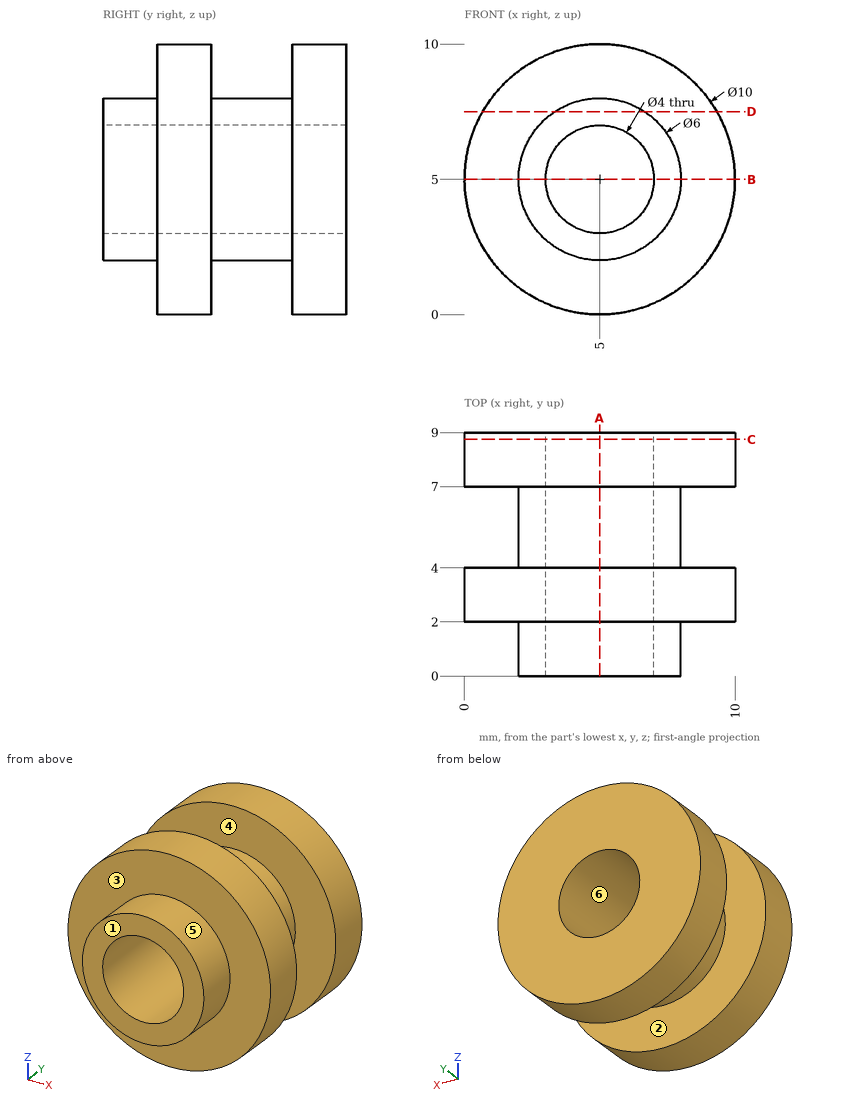
Study the drawing (mm; zero at the part's minimum x, y, z) and answer. A direction names the side the tool comes from. Coordinates: 2 decimals unless noted, no trailing zeros. Write each loop counter-clockwise with the first axis right and the second up, starting at its lowest first coordinate (ties: lowest second). Pieces come first, ordered by that corner, then holes. Notation, with made-up numbers: M -38.5,55.25 L -11.5,55.25 A10 ccw -11.5,67.25 Z; hole C 69,-28.75 d4. An arc over 180 degrees is marked long. Write each question's results on one line, items separated by ' | '.
Item 1: The part is cut by section C-C on y = 8.75. Determine the outline of the cut face in (x, z).
Answer below:
outline: C 5,5 d10; hole C 5,5 d4
Item 2: For a pull along Z with two mould halves and no side action, classify the marked faces 4, 5 and 6 as released by +Z, released by -Z, zero draft, split by the parting line, or undercut.
Answer below:
face 4: zero draft | face 5: split by the parting line | face 6: undercut
Item 3: The part is cut by section D-D on z = 7.5. Determine the outline of the cut face in (x, y).
Answer below:
outline: M 0.67,2 L 3.34,2 L 3.34,0 L 6.66,0 L 6.66,2 L 9.33,2 L 9.33,4 L 6.66,4 L 6.66,7 L 9.33,7 L 9.33,9 L 0.67,9 L 0.67,7 L 3.34,7 L 3.34,4 L 0.67,4 Z
Item 4: Given P1, Ø3, axis at y = 7.5, z = 8.5, coming from the +X side; P2, Ø5, axis at x = 8, y = 3, coming from the +Z side; P3, Ø5, axis at y = 1, z = 1.5, coming from the -X side, each flat-ended and moving along its own axis, determine where each tip first touches the part or whether it passes through.
Answer below:
P1: x = 9.58 | P2: z = 9.97 | P3: x = 0.15
Item 5: The part is cut by section A-A on x = 5. Determine the outline of the cut face in (y, z), and give its area (3 significant figures).
Answer below:
outline: M 0,2 L 2,2 L 2,0 L 4,0 L 4,2 L 7,2 L 7,0 L 9,0 L 9,3 L 0,3 Z; M 0,7 L 9,7 L 9,10 L 7,10 L 7,8 L 4,8 L 4,10 L 2,10 L 2,8 L 0,8 Z | area: 34.0 mm2
Item 6: Which of the six approach directions +Z, -Z, +X, -X, +Y, -Y give full straight-line access (tool end or side, diameter ignored) to the marked faces 1, 2 and 3?
Answer below:
face 1: +Z, -Z, +X, -X, -Y | face 2: none | face 3: -Y
Item 7: The part is cut by section B-B on z = 5. Determine the outline of the cut face in (x, y), and give its area (3 significant figures).
Answer below:
outline: M 0,2 L 2,2 L 2,0 L 3,0 L 3,9 L 0,9 L 0,7 L 2,7 L 2,4 L 0,4 Z; M 7,0 L 8,0 L 8,2 L 10,2 L 10,4 L 8,4 L 8,7 L 10,7 L 10,9 L 7,9 Z | area: 34.0 mm2
Item 8: Consider probe 1 along Y at (x, z) = (2.5, 2.5); probe 2 along X at (y, z) = (4.5, 5); probe 3 along Z at (x, y) = (4.5, 5.25). Determine where each line is inside the solid, lowest interval first. Write a range as [from, to].
Answer below:
probe 1: [2, 4], [7, 9] | probe 2: [2, 3], [7, 8] | probe 3: [2.04, 3.06], [6.94, 7.96]
